The model under review builds one solid part; all positions refer to its coordinate system, in mm. A direction names the side the tool comes from. Give positions to 0.01 mm unless a question says otherwise; leave off trailing zeros. Loops run counter-clockwise (first coordinate to the right, second up) from the corner with the lowest first, then second, coordinate; pieces in that order, holes last. Notation, with made-up numbers: (27, 87) -> (79, 87) arc R11 cw to (79, 104) -> close; hole circle Ø11 at (-37.5, -37.75). An arc over 180 degrees is marked (long way). Write each question's results on one line, items separated by ' | '. Start each with the question number.
Q1. We need section B-B (y = 4.5). Write out the cut boundary in (x, z), plus the area to 4 significant figures.
Q2. Machinability: for faces 1 (the face through (1.5, -65, -36)), 2 (the face through (14.05, -52.27, -116.05)), 3 (the face through (0, 9, -35)), which of the approach directions +Z, -Z, +X, -X, +Y, -Y give a long, thin tool a straight path to every point of the face, cutting with its end or side? Answer none if there is none.
Q3. We need section D-D (y = -43.5). Write out the cut boundary in (x, z).
Q4. Wall thickness on L1, parallel to Y at x = 13.5, z = -73; L2, parallel to Z at x = 20.25, y = -31; L3, parallel to X at y = -56, z = 23: over which ranges is each line inside the solid? List them lowest first. Write a range as [from, to].
Q5. Mouldability with a two-part tool opening along Y and no side actions: class faces 4 (the face through (16, 7.661, -34)), 5 (the face through (28.5, -27, -37)), 6 (the face through (1.5, 13, -34)), 7 (the face through (14, -13, -124.181)) as released by +Y, released by -Y, zero draft, split by the parting line, or undercut.
Q6. We need section A-A (x = 24.5). Write out the cut boundary in (y, z).
Q7. We need section C-C (z = -9). Write out the cut boundary in (x, y), plus the area to 4 significant figures.
Q8. Insertion check: pin 1 Ø4 at (y, z) = (-63, -67) entering from +X; pin 2 Ø12 at (y, z) = (-21, -0.5) entering from -X; pin 3 Ø14 at (x, z) = (14, -37) entering from -Y; pin 4 Ø3 at (y, z) = (-66, -32) entering from +X. Each pin has a flat end and moves straight along its axis. Give the tip position at first contact, or say it passes through.
from build123d import *

# Parameters (mm, degrees)
EXTRUDE_1_DEPTH     = 30
SHELL_1_T           = -1.5
SKETCH_2_W          = 1.5
SKETCH_2_H          = 180
EXTRUDE_2_DEPTH     = 10
SKETCH_5_W          = 1.5
SKETCH_5_H          = 20
EXTRUDE_3_DEPTH     = 10
CUT_EXTRUDE_2_DEPTH = 148.786263339
CHAMFER_1_SIZE      = 3
CHAMFER_2_SIZE      = 3


with BuildPart() as part:
    # 草图1 → 凸台-拉伸1 (new body)
    with BuildSketch(Plane(origin=(0, 0, 0), x_dir=(0, 0, -1), z_dir=(1, 0, 0))):
        with BuildLine():
            Line((-54.319308007, 7.661260091), (125.680691993, 7.661260091))
            Line((125.680691993, 7.661260091), (125.680691993, -32.338739909))
            ThreePointArc((125.680691993, -32.338739909), (116.893895429, -53.551943345), (95.680691993, -62.338739909))
            Line((95.680691993, -62.338739909), (-24.319308007, -62.338739909))
            ThreePointArc((-24.319308007, -62.338739909), (-45.532511442, -53.551943345), (-54.319308007, -32.338739909))
            Line((-54.319308007, -32.338739909), (-54.319308007, 7.661260091))
        make_face()
    extrude(amount=EXTRUDE_1_DEPTH)

    # 抽壳1
    shell_1_openings = [part.faces().sort_by_distance(p)[0] for p in [
        (0, -26.44372844, -35.680691993),
    ]]
    offset(amount=SHELL_1_T, openings=shell_1_openings, kind=Kind.INTERSECTION)

    # 草图2 → 凸台-拉伸2 (add)
    with BuildSketch(Plane(origin=(0, 7.661260091, 0), x_dir=(1, 0, 0), z_dir=(0, 1, 0))):
        with Locations((0.75, 35.680691993)):
            Rectangle(SKETCH_2_W, SKETCH_2_H)
    extrude(amount=EXTRUDE_2_DEPTH)

    # 草图5 → 凸台-拉伸3 (add)
    with BuildSketch(Plane.XZ.offset(62.338739909)):
        with Locations((0.75, -35.680691993)):
            Rectangle(SKETCH_5_W, SKETCH_5_H)
    extrude(amount=EXTRUDE_3_DEPTH)

    # 草图4 → 切除-拉伸2 (cut, through all)
    with BuildSketch(Plane(origin=(1.5, 0, 0), x_dir=(0, 0, -1), z_dir=(1, 0, 0))):
        with BuildLine():
            Line((-29.319308007, 14.411260091), (-19.319308007, 14.411260091))
            ThreePointArc((-19.319308007, 14.411260091), (-17.569308007, 12.661260091), (-19.319308007, 10.911260091))
            Line((-19.319308007, 10.911260091), (-29.319308007, 10.911260091))
            ThreePointArc((-29.319308007, 10.911260091), (-31.069308007, 12.661260091), (-29.319308007, 14.411260091))
        make_face()
        with BuildLine():
            Line((90.680691993, 14.411260091), (100.680691993, 14.411260091))
            ThreePointArc((100.680691993, 14.411260091), (102.430691993, 12.661260091), (100.680691993, 10.911260091))
            Line((100.680691993, 10.911260091), (90.680691993, 10.911260091))
            ThreePointArc((90.680691993, 10.911260091), (88.930691993, 12.661260091), (90.680691993, 14.411260091))
        make_face()
        with BuildLine():
            Line((30.680691993, -65.588739909), (40.680691993, -65.588739909))
            ThreePointArc((40.680691993, -65.588739909), (42.430691993, -67.338739909), (40.680691993, -69.088739909))
            Line((40.680691993, -69.088739909), (30.680691993, -69.088739909))
            ThreePointArc((30.680691993, -69.088739909), (28.930691993, -67.338739909), (30.680691993, -65.588739909))
        make_face()
    extrude(amount=-CUT_EXTRUDE_2_DEPTH, mode=Mode.SUBTRACT)

    # 倒角1
    chamfer_1_edges = [part.edges().sort_by_distance(p)[0] for p in [
        (0.75, 17.661260091, -125.680691993),
        (0.75, 17.661260091, 54.319308007),
    ]]
    chamfer(chamfer_1_edges, length=CHAMFER_1_SIZE)

    # 倒角2
    chamfer_2_edges = [part.edges().sort_by_distance(p)[0] for p in [
        (0.75, -72.338739909, -45.680691993),
        (0.75, -72.338739909, -25.680691993),
    ]]
    chamfer(chamfer_2_edges, length=CHAMFER_2_SIZE)


solid = part.part
Output:
1) outline: (0, -125.68) -> (30, -125.68) -> (30, 54.32) -> (0, 54.32) -> (0, 52.82) -> (28.5, 52.82) -> (28.5, -124.18) -> (0, -124.18) -> close | area: 355.5 mm2
2) face 1: +Z, -Z, +X, -Y | face 2: -X | face 3: +Z, -Z, -X, +Y, -Y
3) outline: (0, -123.53) -> (30, -123.53) -> (30, 52.17) -> (0, 52.17) -> (0, 50.54) -> (28.5, 50.54) -> (28.5, -121.9) -> (0, -121.9) -> close
4) L1: [-62.34, -60.84], [6.16, 7.66] | L2: [-125.68, -124.18], [52.82, 54.32] | L3: [28.5, 30]
5) face 4: released by +Y | face 5: undercut | face 6: zero draft | face 7: undercut
6) outline: (-62.34, -95.68) arc R30 ccw to (-32.34, -125.68) -> (7.66, -125.68) -> (7.66, 54.32) -> (-32.34, 54.32) arc R30 ccw to (-62.34, 24.32) -> close; hole (-60.84, -95.68) arc R28.5 ccw to (-32.34, -124.18) -> (6.16, -124.18) -> (6.16, 52.82) -> (-32.34, 52.82) arc R28.5 ccw to (-60.84, 24.32) -> close
7) outline: (0, -62.34) -> (30, -62.34) -> (30, 7.66) -> (1.5, 7.66) -> (1.5, 17.66) -> (0, 17.66) -> (0, 6.16) -> (28.5, 6.16) -> (28.5, -60.84) -> (0, -60.84) -> close | area: 205.5 mm2
8) pin 1: x = 30 | pin 2: x = 28.5 | pin 3: y = -62.34 | pin 4: x = 1.5
